from build123d import *

# Parameters (mm, degrees)
SKETCH_1_W          = 130
SKETCH_1_H          = 130
SKETCH_1_R          = 4.6
SKETCH_1_R_2        = 55
SKETCH_1_H_2        = 4
EXTRUDE_1_DEPTH     = 5.5
SKETCH_2_R          = 5
EXTRUDE_2_DEPTH     = 11
EXTRUDE_3_DEPTH     = 5
CUT_EXTRUDE_1_DEPTH = 85


with BuildPart() as part:
    # 草图1 → 凸台-拉伸1 (new, symmetric)
    # profile 1 of 4: a face of its own
    with BuildSketch(Plane.XY):
        Rectangle(SKETCH_1_W, SKETCH_1_H)
        with Locations((51.3, -51.3)):
            Circle(SKETCH_1_R, mode=Mode.SUBTRACT)
        with Locations((51.3, 51.3)):
            Circle(SKETCH_1_R, mode=Mode.SUBTRACT)
        with Locations((-51.3, 51.3)):
            Circle(SKETCH_1_R, mode=Mode.SUBTRACT)
        with Locations((0, -0.5)):
            Circle(SKETCH_1_R_2, mode=Mode.SUBTRACT)
        with Locations((-51.3, -51.3)):
            Circle(SKETCH_1_R, mode=Mode.SUBTRACT)
    # profile 2 of 4: a face of its own
    with BuildSketch(Plane.XY):
        with Locations((0, -67)):
            Rectangle(SKETCH_1_W, SKETCH_1_H_2)
    # profile 3 of 4: a face of its own
    with BuildSketch(Plane.XY):
        Polygon((-65, -69), (-65, -65), (-65, 36.950223859), (-79, 24.100911478), (-79, 0), (-79, -69), align=None)
    # profile 4 of 4: a face of its own
    with BuildSketch(Plane.XY):
        Polygon((79, 0), (79, 24.100911478), (65, 36.950223859), (65, -65), (65, -69), (79, -69), align=None)
    extrude(amount=EXTRUDE_1_DEPTH, both=True)

    # 草图2 → 凸台-拉伸2 (add)
    with BuildSketch(Plane.XZ.offset(69)):
        Polygon((-95, -5.543155134), (95, -5.543155134), (95, 94.456844866), (45, 94.456844866), (45, 19.456844866), (-45, 19.456844866), (-45, 94.456844866), (-95, 94.456844866), align=None)
        with Locations(Location((-87, 80.956844866, 0), (0, 0, 270))):
            Circle(SKETCH_2_R, mode=Mode.SUBTRACT)
        with Locations(Location((-87, 10.956844866, 0), (0, 0, 270))):
            Circle(SKETCH_2_R, mode=Mode.SUBTRACT)
        with Locations(Location((87, 10.956844866, 0), (0, 0, 90))):
            Circle(SKETCH_2_R, mode=Mode.SUBTRACT)
        with Locations(Location((87, 80.956844866, 0), (0, 0, 90))):
            Circle(SKETCH_2_R, mode=Mode.SUBTRACT)
    extrude(amount=EXTRUDE_2_DEPTH)

    # 草图3 → 凸台-拉伸3 (add, symmetric)
    with BuildSketch(Plane(origin=(74, 0, 0), x_dir=(0, 0, -1), z_dir=(1, 0, 0))):
        Polygon((-5.5, -5.674954384), (-60.456844866, -69), (-5.5, -69), align=None)
    extrude_3 = extrude(amount=EXTRUDE_3_DEPTH, both=True)

    # 镜向1: 凸台-拉伸3 across plane
    add(extrude_3.mirror(Plane(origin=(0, 0, 0), x_dir=(0, 0, 1), z_dir=(1, 0, 0))))

    # 草图4 → 切除-拉伸1 (cut)
    with BuildSketch(Plane.XY.offset(94.456844866)):
        Polygon((-60, -69), (-45, -74.5), (45, -74.5), (60, -69), align=None)
    extrude(amount=-CUT_EXTRUDE_1_DEPTH, mode=Mode.SUBTRACT)


solid = part.part
Check sheet for the modelled part. Datum: model origin and axes. Units: mm. A direction names the side the tool comes from. Round coordinates to 2 decimals unless told otherwise and drop trailing zeros. Order: outer loops, then holes, each group sorted by start corner. A loop starts at its lowest first (then second) coordinate and runs counter-clockwise, first axis right, second up. Notation, with made-up numbers: M 51,18 L 106,18 A20 ccw 106,30 Z; hole C -18.5,60 d4. An arc over 180 degrees is marked long. One line per item, written item: value. Start each with the question number.
1. Release check for a two-part mould opening along X. For faces 1 (the flat face through (-95, -74, 45)), 2 (the flat face through (-45, -77, 56)), 3 (the flat face through (-1, -74, -5.543)) record: released by +X, released by -X, zero draft, split by the parting line, or undercut.
2. Section check A-A on x = 87. Enter the section's corners in (y, z), and give its area (3 significant figures).
3. Section check C-C on y = -51.3. Enter the section's corners in (x, z), and give its area (3 significant figures).
4. Gauge pin test, flat ends, axial feed: P1, Ø9, axis at y = 56, z = 1, coming from the +X side; P2, Ø4.5, axis at x = -21.5, y = -77.5, coming from the +Z side; P3, Ø1, axis at y = -56.5, z = 24.5, coming from the -X side. Record the tip position at first contact, or that the pin passes through.
5. Section check B-B on z = 69.5. Enter the section's corners in (x, y), and give its area (3 significant figures).
6. Scan lines: line 1 along X through (y, z) = (-67.5, 26.5); line 2 along Z through (x, y) = (-28.5, -54.5); line 3 along Z through (x, y) = (28, -73). Record each from-to range of solid material in increasing order.
7. Access from +Z, -Z, +X, -X, +Y, -Y to the whole of each face (thin tool, end or side, straight path). Record for faces 4 (the flat face through (-65, 51, 0)), 5 (the flat face through (-54, 14, 5.5)), 6 (the flat face through (79, -42, 13)).
8. Section check D-D on x = 0. Enter the section's corners in (y, z).
Results found:
1. face 1: released by -X
1. face 2: undercut
1. face 3: zero draft
2. outline: M -80,-5.54 L -69,-5.54 L -69,5.96 L -80,5.96 Z; M -80,15.96 L -69,15.96 L -69,75.96 L -80,75.96 Z; M -80,85.96 L -69,85.96 L -69,94.46 L -80,94.46 Z
2. area: 880 mm^2
3. outline: M -79,-5.5 L -55.9,-5.5 L -55.9,5.5 L -69,5.5 L -69,45.1 L -79,45.1 Z; M -46.7,-5.5 L -21.08,-5.5 L -21.08,5.5 L -46.7,5.5 Z; M 21.08,-5.5 L 46.7,-5.5 L 46.7,5.5 L 21.08,5.5 Z; M 55.9,-5.5 L 79,-5.5 L 79,45.1 L 69,45.1 L 69,5.5 L 55.9,5.5 Z
3. area: 1,860 mm^2
4. P1: x = 65
4. P2: z = 19.46
4. P3: x = -79
5. outline: M -95,-80 L -45,-80 L -45,-74.5 L -60,-69 L -95,-69 Z; M 45,-80 L 95,-80 L 95,-69 L 60,-69 L 45,-74.5 Z
5. area: 1,020 mm^2
6. line 1: -79 to -69, 69 to 79
6. line 2: -5.5 to 5.5
6. line 3: -5.54 to 9.46
7. face 4: +Z, -Z, -X, +Y
7. face 5: +Z, +Y
7. face 6: +Z, -Z, +X, +Y
8. outline: M -80,-5.54 L -69,-5.54 L -69,-5.5 L -55.5,-5.5 L -55.5,5.5 L -69,5.5 L -69,9.46 L -74.5,9.46 L -74.5,19.46 L -80,19.46 Z; M 54.5,-5.5 L 65,-5.5 L 65,5.5 L 54.5,5.5 Z
